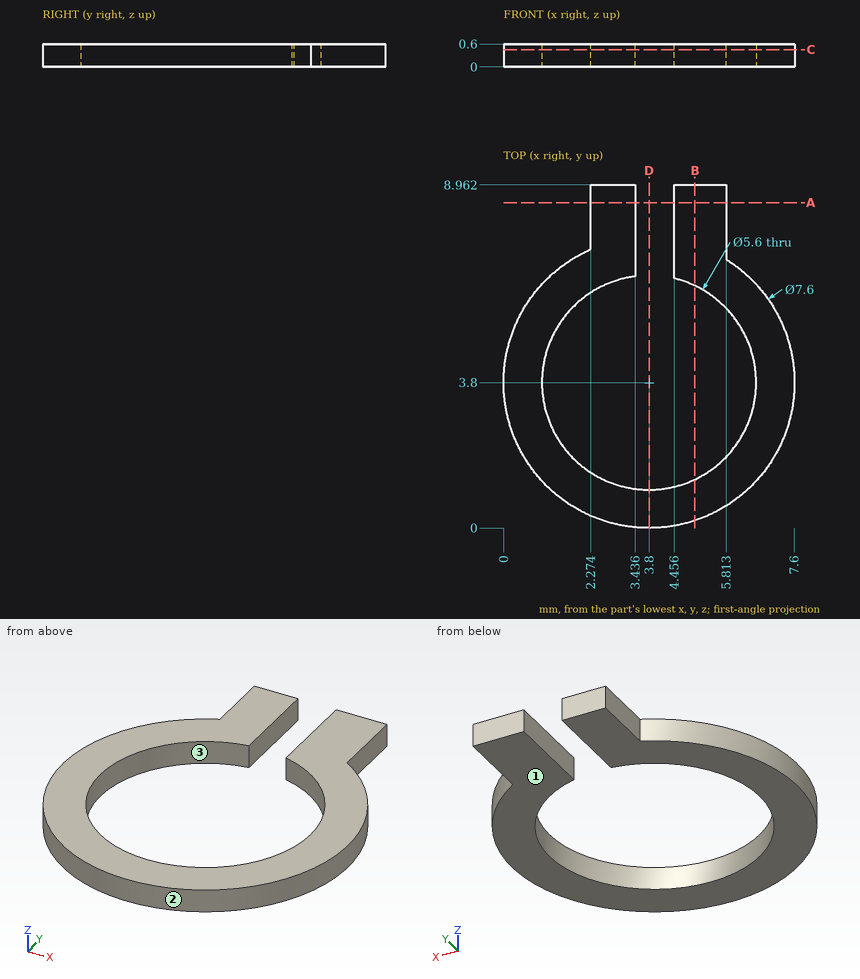
Could you check a few things on this drawing? It's one solid part, dimensions in mm from its lowest x, y, z. Round coordinates to 2 decimals unless told otherwise and drop trailing zeros. Loops run counter-clockwise (first coordinate to the right, second up) from the corner with the lowest first, then second, coordinate; pieces in that order, holes last. Notation, with made-up numbers: (67.5, 31) -> (126.5, 31) arc R25 ccw to (126.5, 48) -> close; hole circle Ø8 at (-6.75, 58). An arc over 180 degrees is marked (long way). One line per item, written item: value. Start each with the question number.
1. If we section it at C-C, the plane z = 0.45: Write out the boundary of the cut face in (x, y) (1 decimal).
2. If we section it at B-B, the plane x = 5: Write out the boundary of the cut face in (y, z) (1 decimal).
3. For pin 1 (1 mm diameter, centred on x = 5.5, y = 4, fed in from +Z), with a flat end and sliding along its axis, tell me the tip position at first contact or that it passes through.
4. If we mould it in two halves opening along Y, with no side actions, what happens to the marked faces 1, 2 and 3? For each: pulls with the +Y half, pulls with the -Y half, needs draft (parallel to the pull), parting line crosses it, or undercut.
5. If we section it at A-A, the plane y = 8.5: Write out the boundary of the cut face in (x, z) (1 decimal).
6. If I drill on probe 1 along X at (y, z) = (3.8, 0.25); probe 2 along X at (y, z) = (8.75, 0.3) (1 decimal); probe 3 along Y at (x, z) = (2.75, 0.4) (1 decimal), over which ranges is the centre line in solid material (lowest first)?
7. If we section it at D-D, the plane x = 3.8: Write out the boundary of the cut face in (y, z).
Calculated:
1. outline: (2.3, 7.3) arc R3.8 ccw (long way) to (5.8, 7) -> (5.8, 9) -> (4.5, 9) -> (4.5, 6.5) arc R2.8 cw (long way) to (3.4, 6.6) -> (3.4, 9) -> (2.3, 9) -> close
2. outline: (0.2, 0) -> (1.3, 0) -> (1.3, 0.6) -> (0.2, 0.6) -> close; (6.3, 0) -> (9, 0) -> (9, 0.6) -> (6.3, 0.6) -> close
3. pin 1: passes through
4. face 1: needs draft
4. face 2: parting line crosses it
4. face 3: undercut
5. outline: (2.3, 0) -> (3.4, 0) -> (3.4, 0.6) -> (2.3, 0.6) -> close; (4.5, 0) -> (5.8, 0) -> (5.8, 0.6) -> (4.5, 0.6) -> close
6. probe 1: x = 0 to 1, 6.6 to 7.6
6. probe 2: x = 2.3 to 3.4, 4.5 to 5.8
6. probe 3: y = 0.1 to 1.2, 6.4 to 9
7. outline: (0, 0) -> (1, 0) -> (1, 0.6) -> (0, 0.6) -> close
